Model file for the job. Use its own axes, mm. A direction names the side the tool comes from. Coordinates: 2 decimals unless noted, no trailing zeros. Write each loop counter-clockwise with the first axis right and the second up, starting at its lowest first coordinate (ties: lowest second). Pieces come first, ordered by that corner, then holes. Notation, with made-up numbers: (21.25, 45.5) -> (60.25, 45.5) arc R15 ccw to (60.25, 69.5) -> close; hole circle Ø11 at (43, 18.5). An arc over 180 degrees is marked (long way). Answer as a JSON object with one key per item and string values. Group by question number.
from build123d import *

# Parameters (mm, degrees)
SKETCH1_R           = 150
BOSS_EXTRUDE1_DEPTH = 10
SKETCH2_R           = 15
BOSS_EXTRUDE2_DEPTH = 46
SKETCH3_R           = 150
BOSS_EXTRUDE3_DEPTH = 10
SKETCH4_R           = 122.5
BOSS_EXTRUDE4_DEPTH = 3.96
CUT_EXTRUDE2_REACH  = 225.371
SKETCH5_R           = 7
CUT_EXTRUDE3_REACH  = 225.371
SKETCH6_R           = 95
CUT_EXTRUDE9_DEPTH  = 10
SKETCH8_R           = 5.5
CUT_EXTRUDE10_DEPTH = 10


with BuildPart() as part:
    # Sketch1 → Boss-Extrude1 (new body)
    with BuildSketch(Plane.XY):
        Circle(SKETCH1_R)
    extrude(amount=BOSS_EXTRUDE1_DEPTH)

    # Sketch2 → Boss-Extrude2 (add)
    with BuildSketch(Plane.XY.offset(10)):
        with Locations((0, 122.5)):
            Circle(SKETCH2_R)
        with Locations((106.088111964, 61.25)):
            Circle(SKETCH2_R)
        with Locations((106.088111964, -61.25)):
            Circle(SKETCH2_R)
        with Locations((0, -122.5)):
            Circle(SKETCH2_R)
        with Locations((-106.088111964, -61.25)):
            Circle(SKETCH2_R)
        with Locations((-106.088111964, 61.25)):
            Circle(SKETCH2_R)
    extrude(amount=BOSS_EXTRUDE2_DEPTH)

    # Sketch3 → Boss-Extrude3 (add)
    with BuildSketch(Plane.XY.offset(56)):
        Circle(SKETCH3_R)
    extrude(amount=BOSS_EXTRUDE3_DEPTH)

    # Sketch4 → Boss-Extrude4 (add)
    with BuildSketch(Plane.XY.offset(66)):
        Circle(SKETCH4_R)
    extrude(amount=BOSS_EXTRUDE4_DEPTH)

    # Cut-Extrude2: up to this face of the body (flat: up to its plane)
    cut_extrude2_end = Plane(part.part.faces().sort_by_distance((0, 0, 69.96))[0])
    # Sketch5 → Cut-Extrude2 (cut, up to the picked face)
    with BuildSketch(Plane(origin=(0, 0, 0), x_dir=(-1, 0, 0), z_dir=(0, 0, -1)), mode=Mode.PRIVATE) as cut_extrude2_sk1:
        with Locations((0, 135)):
            Circle(SKETCH5_R)
    cut_extrude2_tool1 = split(extrude(cut_extrude2_sk1.sketch, amount=-CUT_EXTRUDE2_REACH, mode=Mode.PRIVATE), bisect_by=cut_extrude2_end, keep=Keep.BOTH, mode=Mode.PRIVATE)
    # Sketch5 → Cut-Extrude2 (cut, up to the picked face)
    with BuildSketch(Plane(origin=(0, 0, 0), x_dir=(-1, 0, 0), z_dir=(0, 0, -1)), mode=Mode.PRIVATE) as cut_extrude2_sk2:
        with Locations((116.913429511, 67.5)):
            Circle(SKETCH5_R)
    cut_extrude2_tool2 = split(extrude(cut_extrude2_sk2.sketch, amount=-CUT_EXTRUDE2_REACH, mode=Mode.PRIVATE), bisect_by=cut_extrude2_end, keep=Keep.BOTH, mode=Mode.PRIVATE)
    # Sketch5 → Cut-Extrude2 (cut, up to the picked face)
    with BuildSketch(Plane(origin=(0, 0, 0), x_dir=(-1, 0, 0), z_dir=(0, 0, -1)), mode=Mode.PRIVATE) as cut_extrude2_sk3:
        with Locations((116.913429511, -67.5)):
            Circle(SKETCH5_R)
    cut_extrude2_tool3 = split(extrude(cut_extrude2_sk3.sketch, amount=-CUT_EXTRUDE2_REACH, mode=Mode.PRIVATE), bisect_by=cut_extrude2_end, keep=Keep.BOTH, mode=Mode.PRIVATE)
    # Sketch5 → Cut-Extrude2 (cut, up to the picked face)
    with BuildSketch(Plane(origin=(0, 0, 0), x_dir=(-1, 0, 0), z_dir=(0, 0, -1)), mode=Mode.PRIVATE) as cut_extrude2_sk4:
        with Locations((0, -135)):
            Circle(SKETCH5_R)
    cut_extrude2_tool4 = split(extrude(cut_extrude2_sk4.sketch, amount=-CUT_EXTRUDE2_REACH, mode=Mode.PRIVATE), bisect_by=cut_extrude2_end, keep=Keep.BOTH, mode=Mode.PRIVATE)
    # Sketch5 → Cut-Extrude2 (cut, up to the picked face)
    with BuildSketch(Plane(origin=(0, 0, 0), x_dir=(-1, 0, 0), z_dir=(0, 0, -1)), mode=Mode.PRIVATE) as cut_extrude2_sk5:
        with Locations((-116.913429511, -67.5)):
            Circle(SKETCH5_R)
    cut_extrude2_tool5 = split(extrude(cut_extrude2_sk5.sketch, amount=-CUT_EXTRUDE2_REACH, mode=Mode.PRIVATE), bisect_by=cut_extrude2_end, keep=Keep.BOTH, mode=Mode.PRIVATE)
    # Sketch5 → Cut-Extrude2 (cut, up to the picked face)
    with BuildSketch(Plane(origin=(0, 0, 0), x_dir=(-1, 0, 0), z_dir=(0, 0, -1)), mode=Mode.PRIVATE) as cut_extrude2_sk6:
        with Locations((-116.913429511, 67.5)):
            Circle(SKETCH5_R)
    cut_extrude2_tool6 = split(extrude(cut_extrude2_sk6.sketch, amount=-CUT_EXTRUDE2_REACH, mode=Mode.PRIVATE), bisect_by=cut_extrude2_end, keep=Keep.BOTH, mode=Mode.PRIVATE)
    add(cut_extrude2_tool1.solids().sort_by(Axis((0, 135, 0), (0, 0, 1)))[0], mode=Mode.SUBTRACT)
    add(cut_extrude2_tool2.solids().sort_by(Axis((-116.91343, 67.5, 0), (0, 0, 1)))[0], mode=Mode.SUBTRACT)
    add(cut_extrude2_tool3.solids().sort_by(Axis((-116.91343, -67.5, 0), (0, 0, 1)))[0], mode=Mode.SUBTRACT)
    add(cut_extrude2_tool4.solids().sort_by(Axis((0, -135, 0), (0, 0, 1)))[0], mode=Mode.SUBTRACT)
    add(cut_extrude2_tool5.solids().sort_by(Axis((116.91343, -67.5, 0), (0, 0, 1)))[0], mode=Mode.SUBTRACT)
    add(cut_extrude2_tool6.solids().sort_by(Axis((116.91343, 67.5, 0), (0, 0, 1)))[0], mode=Mode.SUBTRACT)

    # Cut-Extrude3: up to this face of the body (flat: up to its plane)
    cut_extrude3_end = Plane(part.part.faces().sort_by_distance((0, 0, 69.96))[0])
    # Sketch6 → Cut-Extrude3 (cut, up to the picked face)
    with BuildSketch(Plane(origin=(0, 0, 0), x_dir=(-1, 0, 0), z_dir=(0, 0, -1)), mode=Mode.PRIVATE) as cut_extrude3_sk1:
        with Locations(Location((0, 0, 0), (0, 0, 180))):
            Circle(SKETCH6_R)
    cut_extrude3_tool1 = split(extrude(cut_extrude3_sk1.sketch, amount=-CUT_EXTRUDE3_REACH, mode=Mode.PRIVATE), bisect_by=cut_extrude3_end, keep=Keep.BOTH, mode=Mode.PRIVATE)
    add(cut_extrude3_tool1.solids().sort_by(Axis((0, 0, 0), (0, 0, 1)))[0], mode=Mode.SUBTRACT)

    # Sketch7 → Cut-Extrude9 (cut)
    with BuildSketch(Plane(origin=(0, 0, 0), x_dir=(-1, 0, 0), z_dir=(0, 0, -1))):
        with BuildLine():
            ThreePointArc((68.235804385, -68.235804384), (48.250000208, -83.571451345), (24.976038317, -93.211842112))
            ThreePointArc((24.976038317, -93.211842112), (32.789258936, -93.224965512), (39.535945347, -97.165626769))
            ThreePointArc((39.535945347, -97.165626769), (45.088249404, -100.018828425), (51.250848552, -99.023232237))
            ThreePointArc((51.250848552, -99.023232237), (55.75, -96.561832522), (60.131210406, -93.89615293))
            ThreePointArc((60.131210406, -93.89615293), (64.07472157, -89.056983608), (64.379928483, -82.821946418))
            ThreePointArc((64.379928483, -82.821946418), (64.340558994, -75.008813734), (68.235804385, -68.235804384))
        make_face()
    extrude(amount=-CUT_EXTRUDE9_DEPTH, mode=Mode.SUBTRACT)

    # Sketch8 → Cut-Extrude10 (cut)
    with BuildSketch(Plane(origin=(0, 0, 0), x_dir=(-1, 0, 0), z_dir=(0, 0, -1))):
        with Locations((18.817924745, -99.994740903)):
            Circle(SKETCH8_R)
        with Locations((-33.700569576, -96.00694824)):
            Circle(SKETCH8_R)
        with Locations((-77.189023494, -66.294171327)):
            Circle(SKETCH8_R)
        with Locations((-99.994740903, -18.817924745)):
            Circle(SKETCH8_R)
        with Locations((-96.00694824, 33.700569576)):
            Circle(SKETCH8_R)
        with Locations((-66.294171327, 77.189023494)):
            Circle(SKETCH8_R)
        with Locations((-18.817924745, 99.994740903)):
            Circle(SKETCH8_R)
        with Locations((33.700569576, 96.00694824)):
            Circle(SKETCH8_R)
        with Locations((77.189023494, 66.294171327)):
            Circle(SKETCH8_R)
        with Locations((99.994740903, 18.817924745)):
            Circle(SKETCH8_R)
        with Locations((96.00694824, -33.700569576)):
            Circle(SKETCH8_R)
        with Locations((66.294171327, -77.189023494)):
            Circle(SKETCH8_R)
    extrude(amount=-CUT_EXTRUDE10_DEPTH, mode=Mode.SUBTRACT)


solid = part.part
(1) Cut at C-C on z = 5.5. Give the number of separate pieces and of enclosed holes in the cut face, plus the area to 3 significant figures.
(2) Pin check, flat tips, straight feed: pin 1 (2 mm diameter, centred on x = -2.5, z = 60.5, fed in from +Y); pin 2 (12.5 mm diameter, centred on x = 77.19, y = -66.29, fed in from -Z); pin 3 (9 mm diameter, centred on x = -96.01, y = -33.7, fed in from -Z); pin 4 (18 mm diameter, centred on x = 0, y = 135, fed in from +Z). Stop position of each tip, or through.
(3) Cut at B-B on z = 59.5. List the corners of the cut face in (x, y), plus the area to 3 significant figures.
(4) Pull direction X, two halves, no side cores. Call faces 5 (the face through (0.56, -107.51, 32.68)), 6 (the face through (-32.508, 90.638, 4.93)), 7 (the face through (-2, -98, 0)): released by +X, released by -X, zero draft, split by the parting line, or undercut.
(5) Cut at A-A on y = 0. List the corners of the cut face in (x, z), plus the area to 3 significant figures.
(6) Wall check: probe 1 along Z at (x, y) = (65.5, 102); probe 2 along Z at (x, y) = (112.5, 89); probe 3 along Y at (x, z) = (111, 5). Give the ranges that are in metal, low to high.
(7) 3-axis set-ups, long thin cutter, end or side, ignore diameter. For faces 1 (the face through (-23, 123, 66)), 2 (the face through (-20.59, 92.74, 4.93)), 3 (the face through (92.828, 54.239, 32.678)), 4 (the face through (70.348, 80.906, 4.93)): which of +Z, -Z, +X, -X, +Y, -Y reach the whole face in a straight line?
Results found:
{
 "1": {"separate pieces": "1", "enclosed holes": "19", "area": "39,800 mm²"},
 "2": {"pin 1": "stops at y = 149.99", "pin 2": "stops at z = 0", "pin 3": "stops at z = 56", "pin 4": "stops at z = 66"},
 "3": {"outline": "circle Ø300 at (0, 0); hole circle Ø14 at (-116.91, -67.5); hole circle Ø14 at (-116.91, 67.5); hole circle Ø190 at (0, 0); hole circle Ø14 at (0, -135); hole circle Ø14 at (0, 135); hole circle Ø14 at (116.91, -67.5); hole circle Ø14 at (116.91, 67.5)", "area": "41,400 mm²"},
 "4": {"face 5": "split by the parting line", "face 6": "undercut", "face 7": "zero draft"},
 "5": {"outline": "(-150, 0) -> (-95, 0) -> (-95, 10) -> (-150, 10) -> close; (-150, 56) -> (-95, 56) -> (-95, 69.96) -> (-122.5, 69.96) -> (-122.5, 66) -> (-150, 66) -> close; (95, 0) -> (150, 0) -> (150, 10) -> (95, 10) -> close; (95, 56) -> (150, 56) -> (150, 66) -> (122.5, 66) -> (122.5, 69.96) -> (95, 69.96) -> close", "area": "2,420 mm²"},
 "6": {"probe 1": "z = 0 to 10, 56 to 69.96", "probe 2": "z = 0 to 10, 56 to 66", "probe 3": "y = -100.89 to -71.25, -63.75 to 63.75, 71.25 to 100.89"},
 "7": {"face 1": "+Z", "face 2": "+Z, -Z", "face 3": "none", "face 4": "-Z"}
}
